```python
from build123d import *

# Parameters (mm, degrees)
BOSS_EXTRUDE1_DEPTH     = 90
FILLET1_R               = 30
FILLET2_R               = 55
CUT_EXTRUDE1_START      = -90
SKETCH2_R               = 233
CUT_EXTRUDE1_DEPTH      = 180
CUT_EXTRUDE2_DEPTH      = 640.147087923
CUT_EXTRUDE2_DEPTH_BACK = 640.147087923
SKETCH3_W               = 1220
SKETCH3_H               = 21.2
CUT_EXTRUDE3_DEPTH      = 27
MIRROR2_COPY_1_DEPTH    = 27
CUT_EXTRUDE4_DEPTH      = 640.147087923
CUT_EXTRUDE4_DEPTH_BACK = 640.147087923
SKETCH5_R               = 15
SKETCH5_R_2             = 6
CHAMFER1_SIZE           = 3
M36_TAPPED_HOLE1_D      = 32


with BuildPart() as part:
    # Sketch1 → Boss-Extrude1 (new, symmetric)
    with BuildSketch(Plane(origin=(0, 0, 0), x_dir=(0, 0, -1), z_dir=(1, 0, 0))):
        with BuildLine():
            Line((-580, 22), (-252.041663223, 22))
            ThreePointArc((-252.041663223, 22), (0, 253), (252.041663223, 22))
            Line((252.041663223, 22), (580, 22))
            Line((580, 22), (580, -3))
            Line((580, -3), (227.980262304, -3))
            ThreePointArc((227.980262304, -3), (0, 228), (-227.980262304, -3))
            Line((-227.980262304, -3), (-580, -3))
            Line((-580, -3), (-580, 22))
        make_face()
    extrude(amount=BOSS_EXTRUDE1_DEPTH, both=True)

    # Fillet1
    fillet1_edges = [part.edges().sort_by_distance(p)[0] for p in [
        (0, 22, 252.041663223),
        (0, 22, -252.041663223),
    ]]
    fillet(fillet1_edges, radius=FILLET1_R)

    # Fillet2
    fillet2_edges = [part.edges().sort_by_distance(p)[0] for p in [
        (0, -3, -227.980262304),
        (0, -3, 227.980262304),
    ]]
    fillet(fillet2_edges, radius=FILLET2_R)

    # Sketch2 → Cut-Extrude1 (cut)
    with BuildSketch(Plane(origin=(0, 0, 0), x_dir=(0, 0, -1), z_dir=(1, 0, 0)).offset(CUT_EXTRUDE1_START)):
        Circle(SKETCH2_R)
    extrude(amount=CUT_EXTRUDE1_DEPTH, mode=Mode.SUBTRACT)

    # Sketch3 → Cut-Extrude2 (cut, two sides: drawn at the far end of the back side and taken through both)
    with BuildSketch(Plane(origin=(0, 0, 0), x_dir=(0, 0, -1), z_dir=(1, 0, 0)).offset(-CUT_EXTRUDE2_DEPTH_BACK)):
        with Locations((0, -9.4)):
            Rectangle(SKETCH3_W, SKETCH3_H)
    extrude(amount=CUT_EXTRUDE2_DEPTH + CUT_EXTRUDE2_DEPTH_BACK, mode=Mode.SUBTRACT)

    # Sketch4 → Cut-Extrude3 (cut)
    with BuildSketch(Plane(origin=(90, 0, 0), x_dir=(0, 0, -1), z_dir=(1, 0, 0))):
        with BuildLine():
            Line((-598.01008044, 50), (-248.01008044, 50))
            ThreePointArc((-248.01008044, 50), (-252.546221213, 15.14615962), (-252.208247288, -20))
            Line((-252.208247288, -20), (-598.01008044, -20))
            Line((-598.01008044, -20), (-598.01008044, 50))
        make_face()
    cut_extrude3 = extrude(amount=-CUT_EXTRUDE3_DEPTH, mode=Mode.SUBTRACT)

    # Mirror1: Cut-Extrude3 across plane
    add(cut_extrude3.mirror(Plane.XY), mode=Mode.SUBTRACT)

    # Mirror2: Cut-Extrude3 across plane
    add(cut_extrude3.mirror(Plane(origin=(0, 0, 0), x_dir=(0, 0, 1), z_dir=(1, 0, 0))), mode=Mode.SUBTRACT)

    # Mirror2 copy 1 sketch → Mirror2 copy 1 (cut)
    with BuildSketch(Plane.ZY.offset(90)):
        with BuildLine():
            Line((-598.01008044, 50), (-248.01008044, 50))
            ThreePointArc((-248.01008044, 50), (-252.546221213, 15.14615962), (-252.208247288, -20))
            Line((-252.208247288, -20), (-598.01008044, -20))
            Line((-598.01008044, -20), (-598.01008044, 50))
        make_face()
    extrude(amount=-MIRROR2_COPY_1_DEPTH, mode=Mode.SUBTRACT)

    # Sketch5 → Cut-Extrude4 (cut, two sides: drawn at the far end of the back side and taken through both)
    with BuildSketch(Plane(origin=(0, 0, 0), x_dir=(1, 0, 0), z_dir=(0, 1, 0)).offset(-CUT_EXTRUDE4_DEPTH_BACK)):
        with Locations(Location((34, -390, 0), (0, 0, 90))):
            Circle(SKETCH5_R)
        with Locations(Location((34, 390, 0), (0, 0, 90))):
            Circle(SKETCH5_R)
        with Locations(Location((-34, -390, 0), (0, 0, 90))):
            Circle(SKETCH5_R)
        with Locations(Location((-34, 390, 0), (0, 0, 90))):
            Circle(SKETCH5_R)
        with Locations(Location((15, -295, 0), (0, 0, 90))):
            Circle(SKETCH5_R_2)
        with Locations(Location((-15, 295, 0), (0, 0, 90))):
            Circle(SKETCH5_R_2)
    extrude(amount=CUT_EXTRUDE4_DEPTH + CUT_EXTRUDE4_DEPTH_BACK, mode=Mode.SUBTRACT)

    # Chamfer1
    chamfer1_edges = [part.edges().sort_by_distance(p)[0] for p in [
        (-90, 233, 0),
        (90, 233, 0),
    ]]
    chamfer(chamfer1_edges, length=CHAMFER1_SIZE)

    # M36 Tapped Hole1 (through all)
    with Locations(Plane(origin=(0, 1.2, 0), x_dir=(-1, 0, 0), z_dir=(0, -1, 0))):
        with Locations((34, -390), (-34, -390), (-34, 390), (34, 390)):
            Hole(M36_TAPPED_HOLE1_D / 2)


solid = part.part
```
CAD build for the part. Positions are in the model's coordinates, mm. A direction names the side the tool comes from. Round coordinates to 2 decimals unless told otherwise and drop trailing zeros. Order: outer loops, then holes, each group sorted by start corner. A loop starts at its lowest first (then second) coordinate and runs counter-clockwise, first axis right, second up.
Item 1: Probe line 1 along X through (y, z) = (15.25, 390); line 2 along Z through (x, y) = (-34, 11); line 3 along Z through (x, y) = (-34, 17). List the from-to ranges inside material, lowest first.
Item 2: Tool access for faces 1 (the face through (-1, 1.2, 421)), 2 (the face through (-1.26, 9.94, -242.74)), 3 (the face through (1, 22, -427)): list every direction of +Z, -Z, +X, -X, +Y, -Y with a clear straight run to the whole face (end or side of a thin tool).
Item 3: Saw through at A-A on z = 390. Write the cut outline in (x, y), then the cut area to 3 significant figures.
Item 4: Mould opens along Z. For faces 4 (the face through (1, 11, 580)), 5 (the face through (30.53, 11.75, 405.62)), 6 (the face through (-37.47, 11.75, -374.38)), 7 (the face through (90, 240, -1)) say: pulls with the +Z half, pulls with the -Z half, needs draft (parallel to the pull), parting line crosses it, or undercut.
Item 5: Saw through at B-B on x = -34. Write the cut outline in (y, z), then the cut area to 3 significant figures.
Item 6: Pin check, flat tips, straight feed: pin 1 (5 mm diameter, centred on x = -63, z = -147, fed in from -Y); pin 2 (7 mm diameter, centred on x = 15, z = 295, fed in from -Y); pin 3 (13.5 mm diameter, centred on y = 17.5, z = 442.5, fed in from -X); pin 4 (4 mm diameter, centred on x = -49.5, y = 176.5, fed in from +Z). Stop position of each tip, or through.
Reported:
1. line 1: x = -63 to -50, -18 to 18, 50 to 63
1. line 2: z = -580 to -406, -374 to -241.52, 241.52 to 374, 406 to 580
1. line 3: z = -580 to -406, -374 to -235.76, 235.76 to 374, 406 to 580
2. face 1: +Z, -Z, +X, -X, -Y
2. face 2: +X, -X, -Y
2. face 3: -Z, +X, -X, +Y
3. outline: (-63, 1.2) - (-50, 1.2) - (-50, 22) - (-63, 22) - close; (-18, 1.2) - (18, 1.2) - (18, 22) - (-18, 22) - close; (50, 1.2) - (63, 1.2) - (63, 22) - (50, 22) - close
3. area: 1,290 mm2
4. face 4: pulls with the +Z half
4. face 5: undercut
4. face 6: undercut
4. face 7: needs draft
5. outline: (1.2, -580) - (22, -580) - (22, -406) - (1.2, -406) - close; (1.2, -374) - (22, -374) - (22, -278.18) arc R30 cw to (46.49, -248.69) arc R253 ccw to (46.49, 248.69) arc R30 cw to (22, 278.18) - (22, 374) - (1.2, 374) - (1.2, 257.1) arc R55 ccw to (22.23, 231.94) arc R233 cw to (22.23, -231.94) arc R55 ccw to (1.2, -257.1) - close; (1.2, 406) - (22, 406) - (22, 580) - (1.2, 580) - close
5. area: 27,400 mm2
6. pin 1: stops at y = 178.71
6. pin 2: passes through
6. pin 3: stops at x = -63
6. pin 4: stops at z = 183.19
